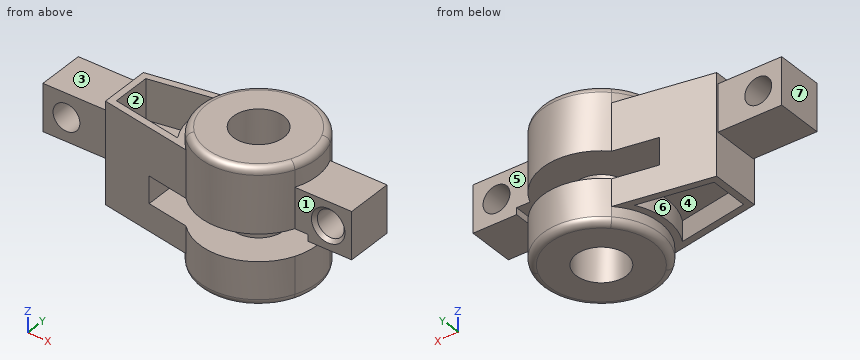
from build123d import *
from build123d.topology import SkipClean

# Parameters (mm, degrees)
BRACKET_SIDE_PROFILE_SKETCH_R = 7.5
BRACKET_BODY_40MM_DEPTH       = 20
TOP_SLOT_CUT_15X19_DEPTH      = 54.124852941
TOP_SLOT_CUT_15X19_DEPTH_BACK = 54.124852941
TOP_SLOT_SKETCH_W             = 45
TOP_SLOT_SKETCH_H             = 8
SIDE_RELIEF_A_CUT_7MM_DEPTH   = 7
SIDE_RELIEF_B_SKETCH_W        = 19
SIDE_RELIEF_B_SKETCH_H        = 14
SIDE_RELIEF_B_CUT_7MM_DEPTH   = 7
LUG_TRIM_A_CUT_5MM_DEPTH      = 5
LUG_START                     = -5
LUG_TRIM_B_CUT_5MM_DEPTH      = 5
HUB_GAP_SKETCH_W              = 19
HUB_GAP_SKETCH_H              = 14
HUB_GAP_CUT_18MM_DEPTH        = 18
RELIEF_STEP_SKETCH_W          = 19
RELIEF_STEP_SKETCH_H          = 14
RELIEF_STEP_CUT_1MM_DEPTH     = 1
WINDOW_START                  = -19
WINDOW_OPENING_CUT_19MM_DEPTH = 19
LUG_HOLE_A_CUT_12MM_DEPTH     = 12
LUG_START_2                   = -6
LUG_HOLE_B_CUT_6MM_DEPTH      = 6
EDGE_FILLET_R2_R              = 2
HUB_BORE_CUT_REACH            = 57.823
HUB_BORE_SKETCH_R             = 4
BORE_CHAMFER_1X45_SIZE        = 1


with BuildPart() as part:
    # Bracket Side Profile Sketch → Bracket Body 40mm (new, symmetric)
    with BuildSketch(Plane.XY):
        with BuildLine():
            Line((-46, -7), (-46, 7))
            Line((-46, 7), (-27, 7))
            Line((-27, 7), (-27, 7.5))
            Line((-27, 7.5), (0.62171804, 12.370454144))
            ThreePointArc((0.62171804, 12.370454144), (16.249720896, 17.195619038), (29.039014932, 7))
            Line((29.039014932, 7), (46, 7))
            Line((46, 7), (46, -7))
            Line((46, -7), (29.039014932, -7))
            ThreePointArc((29.039014932, -7), (16.249720896, -17.195619038), (0.62171804, -12.370454144))
            Line((0.62171804, -12.370454144), (-27, -7.5))
            Line((-27, -7.5), (-27, -7))
            Line((-27, -7), (-46, -7))
        make_face()
        with Locations((13, 0)):
            Circle(BRACKET_SIDE_PROFILE_SKETCH_R, mode=Mode.SUBTRACT)
    extrude(amount=BRACKET_BODY_40MM_DEPTH, both=True)

    # Top Slot Sketch → Top Slot Cut 15x19 (cut, two sides: drawn at the far end of the back side and taken through both)
    with BuildSketch(Plane(origin=(0, 0, 0), x_dir=(1, 0, 0), z_dir=(0, 1, 0)).offset(-TOP_SLOT_CUT_15X19_DEPTH_BACK)):
        with Locations((10.5, 3)):
            Rectangle(TOP_SLOT_SKETCH_W, TOP_SLOT_SKETCH_H)
    extrude(amount=TOP_SLOT_CUT_15X19_DEPTH + TOP_SLOT_CUT_15X19_DEPTH_BACK, mode=Mode.SUBTRACT)

    # Side Relief A Sketch → Side Relief A Cut 7mm (cut)
    with BuildSketch(Plane.XY.offset(20)):
        with BuildLine():
            Line((29.039014932, -7), (46, -7))
            Line((46, -7), (46, 7))
            Line((46, 7), (29.039014932, 7))
            ThreePointArc((29.039014932, 7), (30.5, 0), (29.039014932, -7))
        make_face()
    extrude(amount=-SIDE_RELIEF_A_CUT_7MM_DEPTH, mode=Mode.SUBTRACT)

    # Side Relief B Sketch → Side Relief B Cut 7mm (cut)
    with BuildSketch(Plane.XY.offset(20)):
        with Locations((-36.5, 0)):
            Rectangle(SIDE_RELIEF_B_SKETCH_W, SIDE_RELIEF_B_SKETCH_H)
    extrude(amount=-SIDE_RELIEF_B_CUT_7MM_DEPTH, mode=Mode.SUBTRACT)

    # Lug Trim A Sketch → Lug Trim A Cut 5mm (cut)
    with SkipClean():  # the faces are left unmerged after this step: merging them gives an invalid solid
        with BuildSketch(Plane.XY.offset(20)):
            with BuildLine():
                ThreePointArc((0.62171804, 12.370454144), (-4.5, 0), (0.62171804, -12.370454144))
                Line((0.62171804, -12.370454144), (-27, -7.5))
                Line((-27, -7.5), (-27, 7.5))
                Line((-27, 7.5), (0.62171804, 12.370454144))
            make_face()
        extrude(amount=-LUG_TRIM_A_CUT_5MM_DEPTH, mode=Mode.SUBTRACT)

    # Lug Trim B Sketch → Lug Trim B Cut 5mm (cut)
    with SkipClean():  # the faces are left unmerged after this step: merging them gives an invalid solid
        with BuildSketch(Plane(origin=(0, 0, -20), x_dir=(-1, 0, 0), z_dir=(0, 0, -1)).offset(LUG_START)):
            with BuildLine():
                Line((27, -7.5), (-0.62171804, -12.370454144))
                ThreePointArc((-0.62171804, -12.370454144), (4.5, 0), (-0.62171804, 12.370454144))
                Line((-0.62171804, 12.370454144), (27, 7.5))
                Line((27, 7.5), (27, -7.5))
            make_face()
        extrude(amount=LUG_TRIM_B_CUT_5MM_DEPTH, mode=Mode.SUBTRACT)

    # Hub Gap Sketch → Hub Gap Cut 18mm (cut)
    with SkipClean():  # the faces are left unmerged after this step: merging them gives an invalid solid
        with BuildSketch(Plane(origin=(0, 0, -20), x_dir=(-1, 0, 0), z_dir=(0, 0, -1))):
            with Locations((36.5, 0)):
                Rectangle(HUB_GAP_SKETCH_W, HUB_GAP_SKETCH_H)
        extrude(amount=-HUB_GAP_CUT_18MM_DEPTH, mode=Mode.SUBTRACT)

    # Relief Step Sketch → Relief Step Cut 1mm (cut)
    with SkipClean():  # the faces are left unmerged after this step: merging them gives an invalid solid
        with BuildSketch(Plane.XY.offset(13)):
            with Locations((-36.5, 0)):
                Rectangle(RELIEF_STEP_SKETCH_W, RELIEF_STEP_SKETCH_H)
        extrude(amount=-RELIEF_STEP_CUT_1MM_DEPTH, mode=Mode.SUBTRACT)

    # Window Opening Sketch → Window Opening Cut 19mm (cut)
    with SkipClean():  # the faces are left unmerged after this step: merging them gives an invalid solid
        with BuildSketch(Plane(origin=(0, 0, -20), x_dir=(-1, 0, 0), z_dir=(0, 0, -1)).offset(WINDOW_START)):
            with BuildLine():
                Line((-29.039014932, 7), (-46, 7))
                Line((-46, 7), (-46, -7))
                Line((-46, -7), (-29.039014932, -7))
                ThreePointArc((-29.039014932, -7), (-30.5, 0), (-29.039014932, 7))
            make_face()
        extrude(amount=WINDOW_OPENING_CUT_19MM_DEPTH, mode=Mode.SUBTRACT)

    # Lug Hole A Sketch → Lug Hole A Cut 12mm (cut)
    with SkipClean():  # the faces are left unmerged after this step: merging them gives an invalid solid
        with BuildSketch(Plane.XY.offset(15)):
            with BuildLine():
                Line((-4.017310196, 9.521615078), (-25, 5.821800738))
                Line((-25, 5.821800738), (-25, -5.821800738))
                Line((-25, -5.821800738), (-4.017310196, -9.521615078))
                ThreePointArc((-4.017310196, -9.521615078), (-6.5, 0), (-4.017310196, 9.521615078))
            make_face()
        extrude(amount=-LUG_HOLE_A_CUT_12MM_DEPTH, mode=Mode.SUBTRACT)

    # Lug Hole B Sketch → Lug Hole B Cut 6mm (cut)
    with SkipClean():  # the faces are left unmerged after this step: merging them gives an invalid solid
        with BuildSketch(Plane(origin=(0, 0, -15), x_dir=(-1, 0, 0), z_dir=(0, 0, -1)).offset(LUG_START_2)):
            with BuildLine():
                Line((4.017310196, -9.521615078), (25, -5.821800738))
                Line((25, -5.821800738), (25, 5.821800738))
                Line((25, 5.821800738), (4.017310196, 9.521615078))
                ThreePointArc((4.017310196, 9.521615078), (6.5, 0), (4.017310196, -9.521615078))
            make_face()
        extrude(amount=LUG_HOLE_B_CUT_6MM_DEPTH, mode=Mode.SUBTRACT)

    # Edge Fillet R2
    edge_fillet_r2_edges = [part.edges().sort_by_distance(p)[0] for p in [
        (30.5, 0, -20),
        (30.5, 0, 20),
    ]]
    fillet(edge_fillet_r2_edges, radius=EDGE_FILLET_R2_R)

    # Hub Bore Sketch → Hub Bore Cut (cut, up to next)
    with BuildSketch(Plane(origin=(0, 7, 0), x_dir=(1, 0, 0), z_dir=(0, 1, 0)), mode=Mode.PRIVATE) as hub_bore_cut_sk1:
        with Locations(Location((-39, -5, 0), (0, 0, 180))):
            Circle(HUB_BORE_SKETCH_R)
    hub_bore_cut_tool1 = extrude(hub_bore_cut_sk1.sketch, amount=-HUB_BORE_CUT_REACH, mode=Mode.PRIVATE) & part.part
    # Hub Bore Sketch → Hub Bore Cut (cut, up to next)
    with BuildSketch(Plane(origin=(0, 7, 0), x_dir=(1, 0, 0), z_dir=(0, 1, 0)), mode=Mode.PRIVATE) as hub_bore_cut_sk2:
        with Locations(Location((39, -6, 0), (0, 0, 180))):
            Circle(HUB_BORE_SKETCH_R)
    hub_bore_cut_tool2 = extrude(hub_bore_cut_sk2.sketch, amount=-HUB_BORE_CUT_REACH, mode=Mode.PRIVATE) & part.part
    add(hub_bore_cut_tool1.solids().sort_by_distance((-39, 7, 5))[0], mode=Mode.SUBTRACT)
    add(hub_bore_cut_tool2.solids().sort_by_distance((39, 7, 6))[0], mode=Mode.SUBTRACT)

    # Bore Chamfer 1x45
    bore_chamfer_1x45_edges = [part.edges().sort_by_distance(p)[0] for p in [
        (43, -7, 6),
    ]]
    chamfer(bore_chamfer_1x45_edges, length=BORE_CHAMFER_1X45_SIZE)


solid = part.part
Geometry: final body of the model. Coordinates: model frame, mm. Face numbers are marked on the shaded views. A direction names the side the tool comes from. Give positions to 0.01 mm unless a question says otherwise; leave off trailing zeros. Write each loop counter-clockwise with the first axis right and the second up, starting at its lowest first coordinate (ties: lowest second). Pieces come first, ordered by that corner, then holes. Notation, with made-up numbers: (-9.75, 3) -> (42.25, 3) arc R14 ccw to (42.25, 25) -> close; hole circle Ø6 at (-23.5, 2). An arc over 180 degrees is marked (long way). Answer as a JSON object with one key per item and string values.
1. Cut plane A-A on y = 0. Count the separate pieces of the cut face and the enclosed holes in it, and give its area (3 significant figures).
Ans:
{"separate pieces": "3", "enclosed holes": "2", "area": "1,300 mm^2"}
2. Contact query for flat-ended pins moving along their axis: pin 1 (11 mm diameter, centred on x = -34, z = 5, fed in from +Y); pin 2 (4 mm diameter, centred on y = -3.5, z = -4, fed in from +X); pin 3 (12 mm diameter, centred on y = 9.5, z = -12.5, fed in from +X). Output: stop coordinate, or through.
Ans:
{"pin 1": "stops at y = 7", "pin 2": "stops at x = -12", "pin 3": "stops at x = 30.15"}
3. Cut plane B-B on z = 14. Output: boundary loops of the cut face in (x, y).
Ans:
{"outline": "(-27, -7.5) -> (0.62, -12.37) arc R17.5 ccw (long way) to (0.62, 12.37) -> (-27, 7.5) -> close; hole (-25, -5.82) -> (-4.02, -9.52) arc R19.5 cw to (-4.02, 9.52) -> (-25, 5.82) -> close; hole circle Ø15 at (13, 0)"}
4. Access query for the marked faces 1, 2, 3 and 4. Directions: +Z, -Z, +X, -X, +Y, -Y. A direction counts if a zero-diameter tool reaches every point of the face in a straight line with its end or side. Return the directions, or none.
Ans:
{"face 1": "+Z, -Z, +X, -Y", "face 2": "+Z", "face 3": "+Z, -X, +Y, -Y", "face 4": "-Z"}
5. Mould query, pull axis X, two halves, no side actions, for the marked faces 5, 6 and 7. Classes: pulls with the +X half, pulls with the -X half, needs draft (parallel to the pull), parting line crosses it, or undercut.
Ans:
{"face 5": "needs draft", "face 6": "undercut", "face 7": "pulls with the -X half"}
6. Ray query, probe 1 along Z at (x, y) = (25, 0.5); probe 2 along Z at (x, y) = (-39, -4); probe 3 along X at (y, z) = (0, -11.5). Return the intervals inside material, ascending. Write a range as from..to.
Ans:
{"probe 1": "z = -20..-7, 1..20", "probe 2": "z = -2..1, 9..12", "probe 3": "x = -27..-25, -6.5..5.5, 20.5..30.5"}
7. Cut plane D-D on z = 6. Output: boundary loops of the cut face in (x, y), and give its area (3 significant figures).
Ans:
{"outline": "(-46, -7) -> (-42.87, -7) -> (-42.87, 7) -> (-46, 7) -> close; (-35.13, -7) -> (-27, -7) -> (-27, -7.5) -> (0.62, -12.37) arc R17.5 ccw to (29.04, -7) -> (34, -7) -> (35, -6) -> (35, 7) -> (29.04, 7) arc R17.5 ccw to (0.62, 12.37) -> (-27, 7.5) -> (-27, 7) -> (-35.13, 7) -> close; (43, -6) -> (44, -7) -> (46, -7) -> (46, 7) -> (43, 7) -> close; hole (-25, -5.82) -> (-4.02, -9.52) arc R19.5 cw to (-4.02, 9.52) -> (-25, 5.82) -> close; hole circle Ø15 at (13, 0)", "area": "1,230 mm^2"}
8. Cut plane C-C on x = 39. Output: boundary loops of the cut face in (y, z), and give its area (3 significant figures).
Ans:
{"outline": "(-7, -1) -> (7, -1) -> (7, 2) -> (-6, 2) -> (-7, 1) -> close; (-7, 11) -> (-6, 10) -> (7, 10) -> (7, 13) -> (-7, 13) -> close", "area": "83.0 mm^2"}
